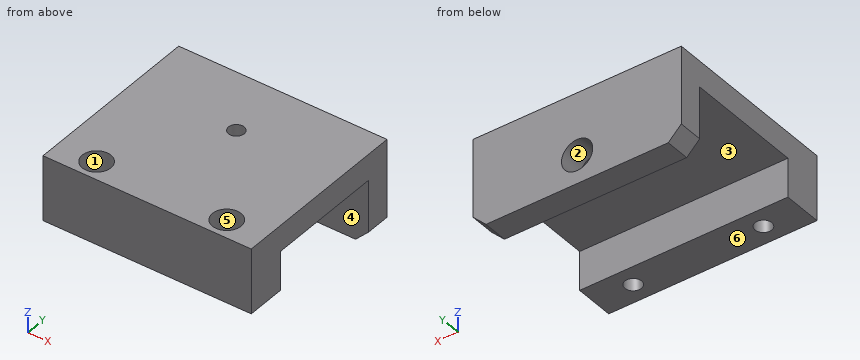
```python
from build123d import *

# Parameters (mm, degrees)
SKETCH_1_W                   = 80
SKETCH_1_H                   = 70
EXTRUDE_1_DEPTH              = 25
SKETCH_2_W                   = 15
SKETCH_2_H                   = 45.5
CUT_EXTRUDE_1_DEPTH          = 109
HOLE_WIZARD_M6_1_D           = 6.4
HOLE_WIZARD_M6_1_CBORE_D     = 11
HOLE_WIZARD_M6_1_CBORE_DEPTH = 6.4
SKETCH_7_R                   = 5.5
CUT_EXTRUDE_3_DEPTH          = 10
SKETCH_8_R                   = 3
CUT_EXTRUDE_4_DEPTH          = 10
SKETCH_9_W                   = 80
SKETCH_9_H                   = 9.5
EXTRUDE_2_DEPTH              = 10
SKETCH_10_R                  = 6
CUT_EXTRUDE_5_DEPTH          = 9.5
CHAMFER_1_SIZE               = 5


with BuildPart() as part:
    # 草图1 → 凸台-拉伸1 (new body)
    with BuildSketch(Plane.XY):
        with Locations((40, 35)):
            Rectangle(SKETCH_1_W, SKETCH_1_H)
    extrude(amount=EXTRUDE_1_DEPTH)

    # 草图2 → 切除-拉伸1 (cut)
    with BuildSketch(Plane(origin=(80, 0, 0), x_dir=(0, 0, -1), z_dir=(1, 0, 0))):
        with Locations((-7.5, 37.75)):
            Rectangle(SKETCH_2_W, SKETCH_2_H)
    extrude(amount=-CUT_EXTRUDE_1_DEPTH, mode=Mode.SUBTRACT)

    # M6 六角凹头螺钉的柱形沉头孔1 (through all)
    with Locations(Plane.XY.offset(25)):
        with Locations((15, 7.5), (65, 7.5)):
            CounterBoreHole(HOLE_WIZARD_M6_1_D / 2, HOLE_WIZARD_M6_1_CBORE_D / 2, HOLE_WIZARD_M6_1_CBORE_DEPTH)

    # 草图7 → 切除-拉伸3 (cut)
    with BuildSketch(Plane.XY.offset(18.6)):
        with Locations((15, 7.5)):
            Circle(SKETCH_7_R)
        with Locations((65, 7.5)):
            Circle(SKETCH_7_R)
    extrude(amount=-CUT_EXTRUDE_3_DEPTH, mode=Mode.SUBTRACT)

    # 草图8 → 切除-拉伸4 (cut)
    with BuildSketch(Plane.XY.offset(25)):
        with Locations((40, 46)):
            Circle(SKETCH_8_R)
    extrude(amount=-CUT_EXTRUDE_4_DEPTH, mode=Mode.SUBTRACT)

    # 草图9 → 凸台-拉伸2 (add)
    with BuildSketch(Plane(origin=(0, 0, 0), x_dir=(-1, 0, 0), z_dir=(0, 0, -1))):
        with Locations((-40, 65.25)):
            Rectangle(SKETCH_9_W, SKETCH_9_H)
    extrude(amount=EXTRUDE_2_DEPTH)

    # 草图10 → 切除-拉伸5 (cut)
    with BuildSketch(Plane(origin=(0, 70, 0), x_dir=(1, 0, 0), z_dir=(0, 1, 0))):
        with Locations(Location((40, -1, 0), (0, 0, 270))):
            Circle(SKETCH_10_R)
    extrude(amount=-CUT_EXTRUDE_5_DEPTH, mode=Mode.SUBTRACT)

    # 倒角1
    chamfer_1_edges = [part.edges().sort_by_distance(p)[0] for p in [
        (80, 65.25, -10),
        (0, 65.25, -10),
    ]]
    chamfer(chamfer_1_edges, length=CHAMFER_1_SIZE)


solid = part.part
```
Build history of the part. All positions in model axes, mm. Face numbers are marked on the shaded views. A direction names the side the tool comes from. Give positions to 0.01 mm unless a question says otherwise; leave off trailing zeros. Loops run counter-clockwise (first coordinate to the right, second up) from the corner with the lowest first, then second, coordinate; pieces in that order, holes last.
Item 1: Flat gauge pins, fed straight in: pin 1 (14.5 mm diameter, centred on x = 65, y = 7.5, fed in from -Z); pin 2 (1.5 mm diameter, centred on x = 26.5, y = 55, fed in from -Z); pin 3 (3.5 mm diameter, centred on x = 15.5, y = 10, fed in from +Z); pin 4 (5.5 mm diameter, centred on x = 40, y = 46, fed in from -Z) (3 decimals). Where does each tip first touch, or does it go through?
Answers follow:
pin 1: stops at z = 0
pin 2: stops at z = 15
pin 3: stops at z = 8.6
pin 4: passes through
Item 2: Pull direction Z, two halves, no side cores. Call the marked faces 1, 2 and 3: released by +Z, released by -Z, zero draft, split by the parting line, or undercut.
Answers follow:
face 1: zero draft
face 2: undercut
face 3: released by -Z
Item 3: Slice it at C-C, the plane y = 46. List the corners of the cut face in (x, z), and give its area (3 significant figures).
Answers follow:
outline: (0, 15) - (37, 15) - (37, 25) - (0, 25) - close; (43, 15) - (80, 15) - (80, 25) - (43, 25) - close
area: 740 mm2
Item 4: Slice it at A-A, the plane z = 10.5. List the corners of the cut face in (x, y).
Answers follow:
outline: (0, 0) - (80, 0) - (80, 15) - (0, 15) - close; (0, 60.5) - (80, 60.5) - (80, 70) - (0, 70) - close; hole circle Ø11 at (15, 7.5); hole circle Ø11 at (65, 7.5)
Item 5: Slice it at B-B, the plane z = 1. List the corners of the cut face in (x, y), and give its area (3 significant figures).
Answers follow:
outline: (0, 0) - (80, 0) - (80, 15) - (0, 15) - close; (0, 60.5) - (34, 60.5) - (34, 70) - (0, 70) - close; (46, 60.5) - (80, 60.5) - (80, 70) - (46, 70) - close; hole circle Ø6.4 at (15, 7.5); hole circle Ø6.4 at (65, 7.5)
area: 1,780 mm2
Item 6: Drill centre lines: line 1 (Y direction, x = 44, z = 13.5); line 2 (X direction, y = 7, z = 7); line 3 (Y direction, x = 15, z = 5). Where is each one in solid material? Low to high.
Answers follow:
line 1: y = 0 to 15, 60.5 to 70
line 2: x = 0 to 11.84, 18.16 to 61.84, 68.16 to 80
line 3: y = 0 to 4.3, 10.7 to 15, 60.5 to 70
Item 7: Which spindle directions (+Z, -Z, +X, -X, +Y, -Y) get a long thin tool onto all of the face, cutting with end or side? Do the marked faces 4, 5 and 6. Say none if no direction does.
Answers follow:
face 4: -Z, +X, -X
face 5: +Z
face 6: -Z, +X, -X, -Y
Item 8: Slice it at D-D, the plane x = 15. List the corners of the cut face in (y, z), and give its area (3 significant figures).
Answers follow:
outline: (0, 0) - (4.3, 0) - (4.3, 8.6) - (2, 8.6) - (2, 25) - (0, 25) - close; (10.7, 0) - (15, 0) - (15, 15) - (60.5, 15) - (60.5, -10) - (70, -10) - (70, 25) - (13, 25) - (13, 8.6) - (10.7, 8.6) - close
area: 927 mm2
